Source: CAD feature listing. Evaluate the final solid. Frame: model axes, mm. A direction names the side the tool comes from. Coordinates: 2 decimals unless noted, no trailing zeros. Order: outer loops, then holes, each group sorted by start corner. A loop starts at its lowest first (then second) coordinate and runs counter-clockwise, first axis right, second up.
```python
from build123d import *

# Parameters (mm, degrees)
BRACKET_BODY_DEPTH = 54
BOSS_SKETCH_R      = 12.5
BOSS_25_DEPTH      = 20
BORE_SKETCH_R      = 8
BORE_16_DEPTH      = 19
HOLE_SKETCH_R      = 6
HOLE_12_DEPTH      = 8


with BuildPart() as part:
    # Bracket Profile Sketch → Bracket Body (new body)
    with BuildSketch(Plane.XY):
        Polygon((0, 0), (0, 30), (54, 30), (54, 22), (8, 22), (8, 0), align=None)
    extrude(amount=BRACKET_BODY_DEPTH)

    # Boss Sketch → Boss Ø25 (add)
    with BuildSketch(Plane(origin=(0, 30, 0), x_dir=(1, 0, 0), z_dir=(0, 1, 0))):
        with Locations(Location((27, -27, 0), (0, 0, 270))):
            Circle(BOSS_SKETCH_R)
    extrude(amount=BOSS_25_DEPTH)

    # Bore Sketch → Bore Ø16 (cut)
    with BuildSketch(Plane(origin=(0, 50, 0), x_dir=(1, 0, 0), z_dir=(0, 1, 0))):
        with Locations(Location((27, -27, 0), (0, 0, 270))):
            Circle(BORE_SKETCH_R)
    extrude(amount=-BORE_16_DEPTH, mode=Mode.SUBTRACT)

    # Hole Sketch → Hole Ø12 (cut)
    with BuildSketch(Plane(origin=(8, 0, 0), x_dir=(0, 0, -1), z_dir=(1, 0, 0))):
        with Locations((-27, 11)):
            Circle(HOLE_SKETCH_R)
    extrude(amount=-HOLE_12_DEPTH, mode=Mode.SUBTRACT)


solid = part.part
```
Q1. Pin query (flat end, axial travel): P1, Ø2, axis at y = 20.5, z = 31.5, coming from the +X side; P2, Ø7, axis at y = 11, z = 27, coming from the -X side; P3, Ø8, axis at x = 34.5, z = 21.5, coming from the -Y side; P4, Ø9.5, axis at x = 27, z = 27, coming from the +Y side. Return the tip coordinate at first contact, or that it passes through.
Solutions:
P1: stops at x = 8
P2: passes through
P3: stops at y = 22
P4: stops at y = 31
Q2. Set-up query: faces 4 (the cylindrical face through (19.394, 39.86, 17.08)), 5 (the cylindrical face through (4.06, 7.35, 31.76)), 6 (the flat face through (8, 11.2, 20.6)). Return all of +Z, -Z, +X, -X, +Y, -Y with unobstructed straight access to the full face (end or side cutting, diameter ignored); none if empty.
Solutions:
face 4: +Y
face 5: +X, -X
face 6: +Z, -Z, +X, -Y
Q3. Section query C-C on x = 27. Output: boundary loops of the cut face in (y, z).
Solutions:
outline: (22, 0) - (30, 0) - (30, 14.5) - (50, 14.5) - (50, 19) - (31, 19) - (31, 35) - (50, 35) - (50, 39.5) - (30, 39.5) - (30, 54) - (22, 54) - close
Q4. Material intervals for line 1 along Y through (x, z) = (4.5, 27); line 2 along X through (y, z) = (42, 27); line 3 along X through (y, z) = (7, 36.5), sorted ascending.
Solutions:
line 1: y = 0 to 5, 17 to 30
line 2: x = 14.5 to 19, 35 to 39.5
line 3: x = 0 to 8
Q5. Pull-direction query (X, two-part tool) for faces 1 (the flat face through (31, 22, 27)), 2 (the cylindrical face through (32.4, 40.6, 21.1)), 3 (the flat face through (54, 26, 27)); classes: pulls with the +X half, pulls with the -X half, needs draft (parallel to the pull), parting line crosses it, or undercut.
Solutions:
face 1: needs draft
face 2: undercut
face 3: pulls with the +X half
Q6. Section query B-B on z = 27. Output: boundary loops of the cut face in (x, y), plus the area to 3 significant figures.
Solutions:
outline: (0, 0) - (8, 0) - (8, 5) - (0, 5) - close; (0, 17) - (8, 17) - (8, 22) - (54, 22) - (54, 30) - (39.5, 30) - (39.5, 50) - (35, 50) - (35, 31) - (19, 31) - (19, 50) - (14.5, 50) - (14.5, 30) - (0, 30) - close
area: 708 mm2
Q7. Section query A-A on y = 11. Output: boundary loops of the cut face in (x, z).
Solutions:
outline: (0, 0) - (8, 0) - (8, 21) - (0, 21) - close; (0, 33) - (8, 33) - (8, 54) - (0, 54) - close
Q8. Section query D-D on z = 9. Output: boundary loops of the cut face in (x, y), plus the area to 3 significant figures.
Solutions:
outline: (0, 0) - (8, 0) - (8, 22) - (54, 22) - (54, 30) - (0, 30) - close
area: 608 mm2
